from build123d import *

# Parameters (mm, degrees)
SKETCH_1_W          = 513
SKETCH_1_H          = 62
EXTRUDE_1_DEPTH     = 15
SHELL_1_T           = 1.5
SKETCH_2_W          = 487
SKETCH_2_H          = 36
CUT_EXTRUDE_1_DEPTH = 2
EXTRUDE_2_DEPTH     = 305
SKETCH_4_W          = 484
SKETCH_4_H          = 33
EXTRUDE_3_DEPTH     = 1.5
SKETCH_6_W          = 108
SKETCH_6_H          = 127
EXTRUDE_4_DEPTH     = 33
SKETCH_7_W          = 105
SKETCH_7_H          = 125.5
CUT_EXTRUDE_2_DEPTH = 33
CUT_EXTRUDE_3_DEPTH = 1.5
SKETCH_9_W          = 286
SKETCH_9_H          = 109
CUT_EXTRUDE_4_DEPTH = 1.5
CUT_EXTRUDE_5_DEPTH = 10
SKETCH_11_R         = 2
CUT_EXTRUDE_6_DEPTH = 400.722716392
FILLET_1_R          = 2


with BuildPart() as part:
    # 草图1 → 凸台-拉伸1 (new body)
    with BuildSketch(Plane.XY):
        Rectangle(SKETCH_1_W, SKETCH_1_H)
    extrude(amount=EXTRUDE_1_DEPTH)

    # 抽壳1 (no face opened: a closed hollow body)
    add(offset(amount=-SHELL_1_T, mode=Mode.PRIVATE), mode=Mode.SUBTRACT)

    # 草图2 → 切除-拉伸1 (cut)
    with BuildSketch(Plane(origin=(0, 0, 0), x_dir=(-1, 0, 0), z_dir=(0, 0, -1))):
        Rectangle(SKETCH_2_W, SKETCH_2_H)
    extrude(amount=-CUT_EXTRUDE_1_DEPTH, mode=Mode.SUBTRACT)

    # 草图3 → 凸台-拉伸2 (add)
    with BuildSketch(Plane(origin=(0, 0, 13.5), x_dir=(-1, 0, 0), z_dir=(0, 0, -1))):
        Polygon((243.5, 18), (-243.5, 18), (-243.5, -18), (-208.5, -18), (-208.5, -16.5), (-242, -16.5), (-242, 16.5), (242, 16.5), (242, -16.5), (208.5, -16.5), (208.5, -18), (243.5, -18), align=None)
    extrude(amount=EXTRUDE_2_DEPTH)

    # 草图4 → 凸台-拉伸3 (add)
    with BuildSketch(Plane(origin=(0, 0, -291.5), x_dir=(-1, 0, 0), z_dir=(0, 0, -1))):
        Rectangle(SKETCH_4_W, SKETCH_4_H)
    extrude(amount=-EXTRUDE_3_DEPTH)

    # 草图6 → 凸台-拉伸4 (add)
    with BuildSketch(Plane.XZ.offset(-16.5)):
        with Locations((151, -226.5)):
            Rectangle(SKETCH_6_W, SKETCH_6_H)
    extrude(amount=EXTRUDE_4_DEPTH)

    # 草图7 → 切除-拉伸2 (cut)
    with BuildSketch(Plane(origin=(0, 18, 0), x_dir=(1, 0, 0), z_dir=(0, 1, 0))):
        with Locations((151, 227.25)):
            Rectangle(SKETCH_7_W, SKETCH_7_H)
    extrude(amount=-CUT_EXTRUDE_2_DEPTH, mode=Mode.SUBTRACT)

    # 草图8 → 切除-拉伸3 (cut)
    with BuildSketch(Plane(origin=(0, 0, -291.5), x_dir=(-1, 0, 0), z_dir=(0, 0, -1))):
        with BuildLine():
            Line((-161, -18), (-161, -3))
            ThreePointArc((-161, -3), (-151, 7), (-141, -3))
            Line((-141, -3), (-141, -18))
            Line((-141, -18), (-161, -18))
        make_face()
    extrude(amount=-CUT_EXTRUDE_3_DEPTH, mode=Mode.SUBTRACT)

    # 草图9 → 切除-拉伸4 (cut)
    with BuildSketch(Plane(origin=(0, 18, 0), x_dir=(1, 0, 0), z_dir=(0, 1, 0))):
        with Locations((-85.5, 81)):
            Rectangle(SKETCH_9_W, SKETCH_9_H)
    extrude(amount=-CUT_EXTRUDE_4_DEPTH, mode=Mode.SUBTRACT)

    # 草图10 → 切除-拉伸5 (cut)
    with BuildSketch(Plane(origin=(0, 18, 0), x_dir=(1, 0, 0), z_dir=(0, 1, 0))):
        with BuildLine():
            Line((-22.5, 153), (37.5, 153))
            ThreePointArc((37.5, 153), (44, 146.5), (37.5, 140))
            Line((37.5, 140), (-22.5, 140))
            ThreePointArc((-22.5, 140), (-29, 146.5), (-22.5, 153))
        make_face()
    extrude(amount=-CUT_EXTRUDE_5_DEPTH, mode=Mode.SUBTRACT)

    # 草图11 → 切除-拉伸6 (cut, through all)
    with BuildSketch(Plane(origin=(0, 0, 13.5), x_dir=(-1, 0, 0), z_dir=(0, 0, -1))):
        with Locations((-16, 11)):
            Circle(SKETCH_11_R)
        with Locations((16, 11)):
            Circle(SKETCH_11_R)
    extrude(amount=-CUT_EXTRUDE_6_DEPTH, mode=Mode.SUBTRACT)

    # 圆角1
    fillet_1_edges = [part.edges().sort_by_distance(p)[0] for p in [
        (-256.5, 0, 15),
        (0, -31, 15),
        (-243.5, 0, 0),
        (0, 18, 0),
        (243.5, 0, 0),
        (226, -18, 0),
        (256.5, 0, 15),
        (-243.5, -18, -145.75),
        (-243.5, 18, -145.75),
        (243.5, 18, -145.75),
        (243.5, -18, -145.75),
        (-226, -18, 0),
        (-243.5, 0, -291.5),
        (243.5, 0, -291.5),
        (0, 31, 15),
        (256.5, -31, 7.5),
        (-256.5, -31, 7.5),
        (-256.5, 31, 7.5),
        (256.5, 31, 7.5),
    ]]
    fillet(fillet_1_edges, radius=FILLET_1_R)


solid = part.part
Verification items for the finished model (mm, model axes). A direction names the side the tool comes from. Give positions to 0.01 mm unless a question says otherwise; leave off trailing zeros. Write each loop counter-clockwise with the first axis right and the second up, starting at its lowest first coordinate (ties: lowest second). Pieces come first, ordered by that corner, then holes.
(1) Material ranges on line 1 (X direction, y = 8, z = -204.5); line 2 (Z direction, x = 163, y = -12); line 3 (Z direction, x = -70.5, y = -9), recorded low to high.
(2) Cross-section at A-A (x = 151). Enter the section's corners in (y, z).
(3) Cross-section at D-D (z = -219). Enter the section's corners in (x, y).
(4) Gauge pin test, flat ends, axial feed: pin 1 (2 mm diameter, centred on x = 150.5, z = -258.5, fed in from +Y); pin 2 (8 mm diameter, centred on x = 124, z = -104, fed in from +Y); pin 3 (3 mm diameter, centred on y = -8, z = -153, fed in from -X). Record the tip position at first contact, or that the pin passes through.
(5) Access from +Z, -Z, +X, -X, +Y, -Y to the whole of each face (thin tool, end or side, straight path). Record for faces 1 (the face through (-243.5, 0, -144)), 2 (the face through (-243.5, 0, 8)), 3 (the face through (205, 0, -227)), 4 (the face through (151, 7, -291)).
(6) Cross-section at B-B (z = -117.5). Enter the section's corners in (x, y).
(7) Cross-section at C-C (x = 84.5). Enter the section's corners in (y, z).
(8) Mould release check, pull along Y, two halves, no side actions. Record for faces 5 (the face through (-4, -31, 6)), 6 (the face through (-4, 31, 6)), 7 (the face through (-4, 21, 0)), 8 (the face through (-226, -18, 8)): +Y half, -Y half, draft (parallel to the pull), parting line (faces both ways), or undercut.
Worked out:
1. line 1: x = -243.5 to -242, 97 to 98.5, 203.5 to 205, 242 to 243.5
1. line 2: z = -291.5 to -290, -164.5 to -163, 13.5 to 15
1. line 3: z = -291.5 to -290, 13.5 to 15
2. outline: (-31, 0) - (-18, 0) - (-18, 1.5) - (-29.5, 1.5) - (-29.5, 13.5) - (16.5, 13.5) - (16.5, -163) - (-16.5, -163) - (-16.5, -290) - (-15, -290) - (-15, -164.5) - (18, -164.5) - (18, -2) arc R2 cw to (20, 0) - (31, 0) - (31, 13) arc R2 ccw to (29, 15) - (-29, 15) arc R2 ccw to (-31, 13) - close; (7, -291.5) - (18, -291.5) - (18, -290) - (7, -290) - close; hole (18, 1.5) - (29.5, 1.5) - (29.5, 13.5) - (18, 13.5) - close
3. outline: (-243.5, -16) arc R2 ccw to (-241.5, -18) - (-208.5, -18) - (-208.5, -16.5) - (-242, -16.5) - (-242, 16.5) - (97, 16.5) - (97, -16.5) - (205, -16.5) - (205, 16.5) - (242, 16.5) - (242, -16.5) - (208.5, -16.5) - (208.5, -18) - (241.5, -18) arc R2 ccw to (243.5, -16) - (243.5, 16) arc R2 ccw to (241.5, 18) - (203.5, 18) - (203.5, -15) - (98.5, -15) - (98.5, 18) - (-241.5, 18) arc R2 ccw to (-243.5, 16) - close
4. pin 1: stops at y = -15
4. pin 2: stops at y = 18
4. pin 3: stops at x = -243.5
5. face 1: -Z, -X, +Y, -Y
5. face 2: none
5. face 3: -Y
5. face 4: -Z, -Y
6. outline: (-243.5, -16) arc R2 ccw to (-241.5, -18) - (-208.5, -18) - (-208.5, -16.5) - (-242, -16.5) - (-242, 16.5) - (-228.5, 16.5) - (-228.5, 18) - (-241.5, 18) arc R2 ccw to (-243.5, 16) - close; (57.5, 16.5) - (242, 16.5) - (242, -16.5) - (208.5, -16.5) - (208.5, -18) - (241.5, -18) arc R2 ccw to (243.5, -16) - (243.5, 16) arc R2 ccw to (241.5, 18) - (57.5, 18) - close
7. outline: (-31, 0) - (-18, 0) - (-18, 1.5) - (-29.5, 1.5) - (-29.5, 13.5) - (16.5, 13.5) - (16.5, -290) - (-16.5, -290) - (-16.5, -291.5) - (18, -291.5) - (18, -2) arc R2 cw to (20, 0) - (31, 0) - (31, 13) arc R2 ccw to (29, 15) - (-29, 15) arc R2 ccw to (-31, 13) - close; hole (18, 1.5) - (29.5, 1.5) - (29.5, 13.5) - (18, 13.5) - close
8. face 5: -Y half
8. face 6: +Y half
8. face 7: draft
8. face 8: undercut
